from build123d import *

# Parameters (mm, degrees)
BOSS_EXTRUDE1_DEPTH   = 100
SKETCH3_R             = 1
CUT_EXTRUDE2_DEPTH    = 10
LPATTERN1_COUNT       = 2
LPATTERN1_PITCH       = 80
M3_TAPPED_HOLE1_D     = 2.5
M3_TAPPED_HOLE1_DEPTH = 7.5
M3_TAPPED_HOLE1_TIP   = 0.751075774
CHAMFER2_SIZE         = 0.5
SKETCH6_W             = 85.5
SKETCH6_H             = 68.5
CUT_EXTRUDE4_DEPTH    = 10
CHAMFER3_SIZE         = 30
FILLET1_R             = 3
SKETCH7_R             = 4
CUT_EXTRUDE5_DEPTH    = 10
SKETCH9_W             = 119.5
SKETCH9_H             = 50
BOSS_EXTRUDE2_DEPTH   = 3
SKETCH5_R             = 2.5
CUT_EXTRUDE3_DEPTH    = 10
CHAMFER4_SIZE         = 3
CHAMFER5_SIZE         = 30
M3_TAPPED_HOLE2_D     = 2.5
M3_TAPPED_HOLE2_DEPTH = 7.5
M3_TAPPED_HOLE2_TIP   = 0.751075774
M3_TAPPED_HOLE3_D     = 2.5
M3_TAPPED_HOLE3_DEPTH = 7.5
M3_TAPPED_HOLE3_TIP   = 0.751075774


with BuildPart() as part:
    # Sketch1 → Boss-Extrude1 (new body)
    with BuildSketch(Plane(origin=(0, 0, 0), x_dir=(1, 0, 0), z_dir=(0, 1, 0))):
        Polygon((0, 120), (-34.202014333, 213.969262079), (-37.021092195, 212.943201649), (-3, 119.471019058), (-3, 0), (0, 0), align=None)
    extrude(amount=BOSS_EXTRUDE1_DEPTH)

    # Sketch3 → Cut-Extrude2 (cut)
    with BuildSketch(Plane(origin=(35.748178719, 0, -13.011272983), x_dir=(0.3420201433256699, 0, 0.939692620785908), z_dir=(-0.9396926207859081, 0, 0.3420201433256699))):
        with Locations((-202.763114494, 86)):
            Circle(SKETCH3_R)
        with Locations((-202.763114494, 14)):
            Circle(SKETCH3_R)
    cut_extrude2 = extrude(amount=-CUT_EXTRUDE2_DEPTH, mode=Mode.SUBTRACT)

    # LPattern1: Cut-Extrude2 ×2
    with Locations(*[Vector(0.3420201433256699, 0, 0.939692620785908) * (i * LPATTERN1_PITCH) for i in range(1, LPATTERN1_COUNT)]):
        add(cut_extrude2, mode=Mode.SUBTRACT)

    # M3 Tapped Hole1
    with Locations(Plane(origin=(-30.781812899, 86, -204.572335871), x_dir=(0.342020143326, 0, 0.939692620786), z_dir=(0.939692620786, 0, -0.342020143326))):
        with Locations((0, 0), (0, 72), (80, 72), (80, 0)):
            Hole(M3_TAPPED_HOLE1_D / 2, depth=M3_TAPPED_HOLE1_DEPTH)
            with Locations((0, 0, -(M3_TAPPED_HOLE1_DEPTH + M3_TAPPED_HOLE1_TIP / 2))):  # 118° drill point
                Cone(0, M3_TAPPED_HOLE1_D / 2, M3_TAPPED_HOLE1_TIP, mode=Mode.SUBTRACT)

    # Chamfer2
    chamfer2_edges = [part.edges().sort_by_distance(p)[0] for p in [
        (-2.992676254, 86, -128.222310432),
        (-2.992676254, 14, -128.222310432),
        (-30.35428772, 14, -203.397720095),
        (-30.35428772, 86, -203.397720095),
    ]]
    chamfer(chamfer2_edges, length=CHAMFER2_SIZE)

    # Sketch6 → Cut-Extrude4 (cut)
    with BuildSketch(Plane.ZY.offset(3)):
        with Locations((-42.75, 65.75)):
            Rectangle(SKETCH6_W, SKETCH6_H)
    extrude(amount=-CUT_EXTRUDE4_DEPTH, mode=Mode.SUBTRACT)

    # Chamfer3
    chamfer3_edges = [part.edges().sort_by_distance(p)[0] for p in [
        (-1.5, 100, -85.5),
    ]]
    chamfer(chamfer3_edges, length=CHAMFER3_SIZE)

    # Fillet1
    fillet1_edges = [part.edges().sort_by_distance(p)[0] for p in [
        (-1.5, 31.5, -85.5),
    ]]
    fillet(fillet1_edges, radius=FILLET1_R)

    # Sketch7 → Cut-Extrude5 (cut)
    with BuildSketch(Plane(origin=(35.748178719, 0, -13.011272983), x_dir=(0.3420201433256699, 0, 0.939692620785908), z_dir=(-0.9396926207859081, 0, 0.3420201433256699))):
        with Locations((-176.263114494, 50)):
            Circle(SKETCH7_R)
    extrude(amount=-CUT_EXTRUDE5_DEPTH, mode=Mode.SUBTRACT)

    # Sketch9 → Boss-Extrude2 (add)
    with BuildSketch(Plane.ZY.offset(3)):
        with Locations((-59.75, -25)):
            Rectangle(SKETCH9_W, SKETCH9_H)
    extrude(amount=-BOSS_EXTRUDE2_DEPTH)

    # Sketch5 → Cut-Extrude3 (cut)
    with BuildSketch(Plane.ZY.offset(3)):
        with Locations((-8, 21.5)):
            Circle(SKETCH5_R)
        with Locations((-8, -42)):
            Circle(SKETCH5_R)
        with Locations((-66, 21.5)):
            Circle(SKETCH5_R)
        with Locations((-66, -42)):
            Circle(SKETCH5_R)
    extrude(amount=-CUT_EXTRUDE3_DEPTH, mode=Mode.SUBTRACT)

    # Chamfer4
    chamfer4_edges = [part.edges().sort_by_distance(p)[0] for p in [
        (-1.5, 31.5, 0),
        (-35.611553264, 100, -213.456231864),
        (-35.611553264, 0, -213.456231864),
        (-1.5, -50, 0),
    ]]
    chamfer(chamfer4_edges, length=CHAMFER4_SIZE)

    # Chamfer5
    chamfer5_edges = [part.edges().sort_by_distance(p)[0] for p in [
        (-1.5, -50, -119.5),
    ]]
    chamfer(chamfer5_edges, length=CHAMFER5_SIZE)

    # M3 Tapped Hole2
    with Locations(Plane(origin=(35.748178719, 0, -13.011272983), x_dir=(0.3420201433256699, 0, 0.939692620785908), z_dir=(-0.9396926207859081, 0, 0.3420201433256699))):
        with Locations((-117.763114494, 50)):
            Hole(M3_TAPPED_HOLE2_D / 2, depth=M3_TAPPED_HOLE2_DEPTH)
            with Locations((0, 0, -(M3_TAPPED_HOLE2_DEPTH + M3_TAPPED_HOLE2_TIP / 2))):  # 118° drill point
                Cone(0, M3_TAPPED_HOLE2_D / 2, M3_TAPPED_HOLE2_TIP, mode=Mode.SUBTRACT)

    # M3 Tapped Hole3
    with Locations(Plane.ZY.offset(3)):
        with Locations((-107.5, -2)):
            Hole(M3_TAPPED_HOLE3_D / 2, depth=M3_TAPPED_HOLE3_DEPTH)
            with Locations((0, 0, -(M3_TAPPED_HOLE3_DEPTH + M3_TAPPED_HOLE3_TIP / 2))):  # 118° drill point
                Cone(0, M3_TAPPED_HOLE3_D / 2, M3_TAPPED_HOLE3_TIP, mode=Mode.SUBTRACT)


solid = part.part
Check sheet for the modelled part. Datum: model origin and axes. Units: mm. A direction names the side the tool comes from. Give positions to 0.01 mm unless a question says otherwise; leave off trailing zeros. Write each loop counter-clockwise with the first axis right and the second up, starting at its lowest first coordinate (ties: lowest second). Pieces come first, ordered by that corner, then holes. Notation, with made-up numbers: (-4.5, 24.25) -> (33.5, 24.25) arc R11 ccw to (33.5, 36.25) -> close; hole circle Ø7 at (56.25, 8). An arc over 180 degrees is marked (long way). Write item = value, one per line.
Item 1: Scan lines: probe 1 along Y at (x, z) = (-1.85, -66); probe 2 along X at (y, z) = (5, -35); probe 3 along X at (y, z) = (69.5, -157.5). Record each from-to range of solid material in increasing order. Write a range as from..to.
Output:
probe_1 = -50..-44.5, -39.5..19, 24..31.5
probe_2 = -3..0
probe_3 = -16.84..-13.65
Item 2: Tool access check on faces 1 (the cylindrical face through (-24.233, 47.566, -182.133)), 2 (the flat face through (-3, 9, -74)). Record the directions out of +Z, -Z, +X, -X, +Y, -Y that give a thin tool (end or side, any length) a straight path to the whole face; none if there is none.
Output:
face_1 = none
face_2 = +Z, -X, +Y, -Y
Item 3: Gauge pin test, flat ends, axial feed: pin 1 (0.9 mm diameter, centred on x = -1.5, y = -7, fed in from -Z); pin 2 (6.5 mm diameter, centred on y = -42, z = -66, fed in from -X); pin 3 (6.5 mm diameter, centred on y = 21.5, z = -8, fed in from +X); pin 4 (0.9 mm diameter, centred on x = -1, y = 55.5, fed in from +Z). Record the tip position at first contact, or that the pin passes through.
Output:
pin_1 = -119.5
pin_2 = -3
pin_3 = 0
pin_4 = -85.5
Item 4: Sectioned sample at A-A on y = -42. Record the boundary of the cut face in (x, z).
Output:
outline = (-3, -97.5) -> (0, -97.5) -> (0, -68.5) -> (-3, -68.5) -> close; (-3, -63.5) -> (0, -63.5) -> (0, -10.5) -> (-3, -10.5) -> close; (-3, -5.5) -> (0, -5.5) -> (0, 0) -> (-3, 0) -> close
Item 5: Sectioned sample at C-C on z = -78.5. Record the boundary of the cut face in (x, y), and give its area (4 significant figures).
Output:
outline = (-3, -50) -> (0, -50) -> (0, 31.5) -> (-3, 31.5) -> close
area = 244.5 mm^2
Item 6: Sectioned sample at D-D on x = -9. Record the boundary of the cut face in (y, z).
Output:
outline = (0, -144.73) -> (100, -144.73) -> (100, -135.96) -> (0, -135.96) -> close
Item 7: Sectioned sample at B-B on y = 9.5. Record the boundary of the cut face in (x, z), and give its area (3 significant figures).
Output:
outline = (-37.02, -212.94) -> (-34.2, -213.97) -> (0, -120) -> (0, 0) -> (-3, 0) -> (-3, -119.47) -> close
area = 658 mm^2
Item 8: Release check for a two-part mould opening along Y. For faces 3 (the cylindrical face through (-1.52, -44.44, -8.54)), 4 (the flat face through (-1.5, 84.8, -100.3)), 5 (the flat face through (-16.862, 49.3, -166.327)), 6 (the flat face through (-1.5, -34.8, -104.7)) record: +Y half, -Y half, draft (parallel to the pull), parting line (faces both ways), or undercut.
Output:
face_3 = undercut
face_4 = +Y half
face_5 = draft
face_6 = -Y half
